Design review of the part shown in the three views and the two pictorial views. Dimensions are in mm from the part's minimum x, y and z. A direction names the side the tool comes from. Coordinates: 2 decimals unless noted, no trailing zeros. Loops run counter-clockwise (first coordinate to the right, second up) from the corner with the lowest first, then second, coordinate; pieces in that order, holes last.
Q1. Draft analysis for pull direction Y (two halves, no side actions). For the marked faces 3, 4 and 5, state which applies: released by +Y, released by -Y, zero draft, split by the parting line, or undercut.
Q2. For P1, Ø5, axis at y = 7, z = 7, coming from the +X side; P2, Ø4, axis at x = 9, y = 3, coming from the -Z side; P3, Ø3, axis at x = 10, z = 4.5, coming from the -Y side; P4, Ø1, axis at x = 6.5, z = 7.5, coming from the -Y side, all flat-tipped, find the tip position at first contact; note any pin that passes through.
Q3. Wall thickness on probe 1 along Z at (x, y) = (3.5, 7); probe 2 along X at (y, z) = (4.75, 1): over which ranges is each line inside the solid? List them lowest first.
Q4. Add section A-A on z = 7. Give the boundary of the cut face in (x, y), and give its area (3 significant figures).
Q5. Add section C-C on x = 3.75. Give the boundary of the cut face in (y, z).
Q6. Machinability: for the marked faces 1 and 2, which of the approach directions +Z, -Z, +X, -X, +Y, -Y give a long, thin tool a straight path to every point of the face, cutting with its end or side? Answer none if there is none.
Q7. Add section D-D on x = 10.25. Give the boundary of the cut face in (y, z), and give its area (3 significant figures).
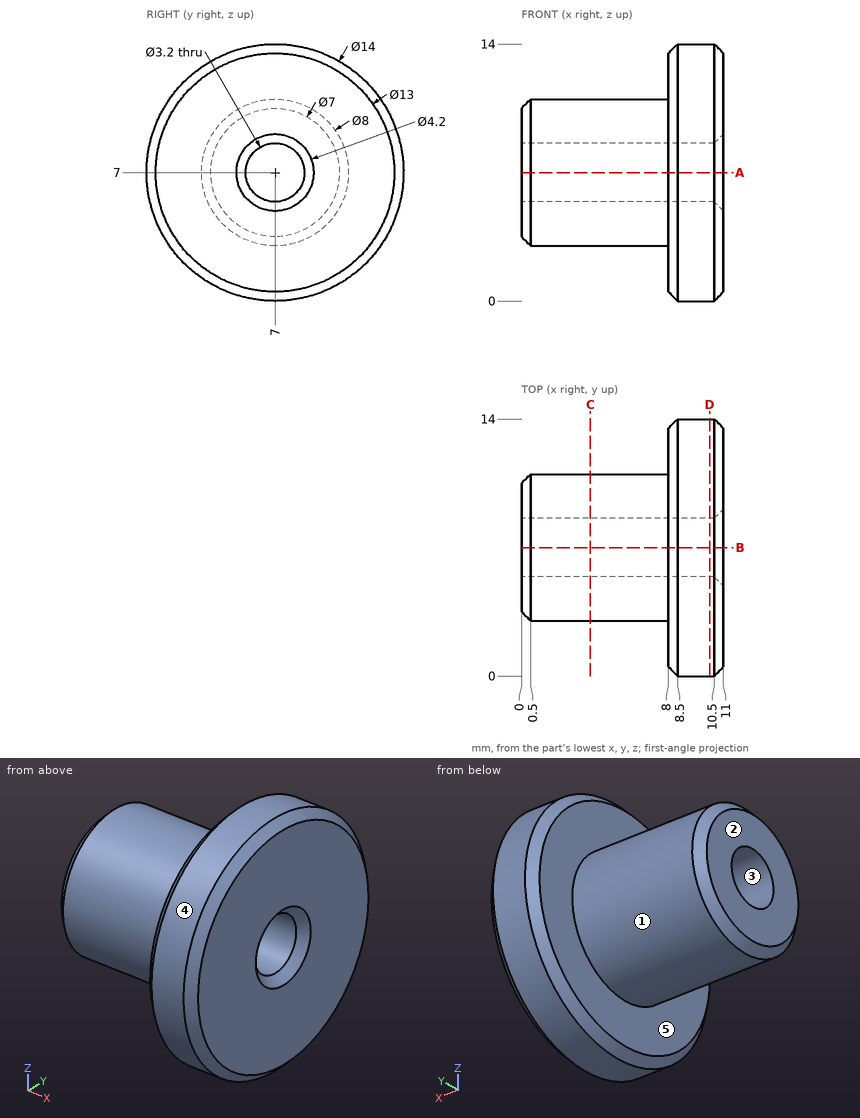
Entries:
1. face 3: undercut
1. face 4: split by the parting line
1. face 5: zero draft
2. P1: stops at x = 11
2. P2: stops at z = 0.29
2. P3: stops at y = 0.07
2. P4: stops at y = 3
3. probe 1: z = 3 to 5.4, 8.6 to 11
3. probe 2: x = 8 to 11
4. outline: (0, 3.5) - (0.5, 3) - (8, 3) - (8, 0.5) - (8.5, 0) - (10.5, 0) - (11, 0.5) - (11, 4.9) - (10.5, 5.4) - (0, 5.4) - close; (0, 8.6) - (10.5, 8.6) - (11, 9.1) - (11, 13.5) - (10.5, 14) - (8.5, 14) - (8, 13.5) - (8, 11) - (0.5, 11) - (0, 10.5) - close
4. area: 69.8 mm2
5. outline: circle Ø8 at (7, 7); hole circle Ø3.2 at (7, 7)
6. face 1: -X
6. face 2: +Z, -Z, -X, +Y, -Y
7. outline: circle Ø14 at (7, 7); hole circle Ø3.2 at (7, 7)
7. area: 146 mm2
